Part model, mm, in its own coordinate system. A direction names the side the tool comes from. Coordinates: 2 decimals unless noted, no trailing zeros. Order: outer loops, then holes, each group sorted by start corner. A loop starts at its lowest first (then second) coordinate and runs counter-clockwise, first axis right, second up. Notation, with made-up numbers: (63, 75) - (73, 75) arc R19 ccw to (73, 94) - close; hole circle Ø10 at (11.25, 12.5). An arc over 180 degrees is marked (long way). Use a Markdown table: item, result. Add a question column.
1) Saw through at B-B on z = -28.5. List the corners of the cut face in (x, y), then the cut area to 3 significant figures.
2) Drop flat-ended pins along their axis: P1, Ø14.5, axis at x = 54.5, y = -42.5, coming from the -Z side; P2, Ø12, axis at y = -70.5, z = -56.5, coming from the -X side; P3, Ø12, axis at y = -11.5, z = -26, coming from the -X side. Give the stop position or say it passes through.
3) Saw through at D-D on x = 12. List the corners of the cut face in (y, z), then the cut area to 3 significant figures.
4) Tool access for faces 1 (the face through (37.1, -19.76, -46.64)), 2 (the face through (49, 0, -37)), 3 (the face through (90, -142, 10)), 4 (the face through (0, -74, 10)), 5 (the face through (90, -20, -45)): list every direction of +Z, -Z, +X, -X, +Y, -Y with a clear straight run to the whole face (end or side of a thin tool).
5) Two-plate mould, pull along Y, no slides. Class faces 6 (the face through (10, -20, -45)), 7 (the face through (49.93, -95.495, -46.644)), 8 (the face through (50, -40, 0)): +Y half, -Y half, draft (parallel to the pull), parting line (faces both ways), or undercut.
6) Saw through at A-A on y = -138.5. List the corners of the cut face in (x, z).
7) Saw through at C-C on y = -30. List the corners of the cut face in (x, z), then the cut area to 3 significant figures.
8) Wall check: L1, parallel to X at y = -6, z = -82; L2, parallel to Z at x = 83, y = -73; L3, parallel to Y at x = 49, z = -75.5. Give the ranges that are in metal, low to high. Write a range as [from, to].
```python
from build123d import *

# Parameters (mm, degrees)
BASE_PLATE_20MM_DEPTH   = 20
BLOCK_92MM_DEPTH        = 92
RELIEF_CUT_SKETCH_R     = 24
RELIEF_CUT_DEPTH        = 92
GUSSET_100MM_DEPTH      = 100
GUSSET_TRIM_CUT_1_DEPTH = 45
GUSSET_TRIM_CUT_2_DEPTH = 45


with BuildPart() as part:
    # Base Plate Sketch → Base Plate 20mm (new body)
    with BuildSketch(Plane.XY):
        Polygon((0, 0), (100, 0), (100, -150), (90, -150), (90, -134), (10, -134), (10, -150), (0, -150), align=None)
    extrude(amount=BASE_PLATE_20MM_DEPTH)

    # Block Sketch → Block 92mm (add)
    with BuildSketch(Plane(origin=(0, 0, 0), x_dir=(-1, 0, 0), z_dir=(0, 0, -1))):
        with BuildLine():
            Line((-10, -40), (-10, 0))
            Line((-10, 0), (-90, 0))
            Line((-90, 0), (-90, -40))
            ThreePointArc((-90, -40), (-50, -80), (-10, -40))
        make_face()
    extrude(amount=BLOCK_92MM_DEPTH)

    # Relief Cut Sketch → Relief Cut (cut)
    with BuildSketch(Plane(origin=(0, 0, -92), x_dir=(-1, 0, 0), z_dir=(0, 0, -1))):
        with Locations((-50, -40)):
            Circle(RELIEF_CUT_SKETCH_R)
    extrude(amount=-RELIEF_CUT_DEPTH, mode=Mode.SUBTRACT)

    # Gusset Sketch → Gusset 100mm (add)
    with BuildSketch(Plane.ZY):
        Polygon((-92, -80), (0, -111.42938948), (0, -79.30503211), align=None)
    extrude(amount=-GUSSET_100MM_DEPTH)

    # Gusset Trim Sketch 1 → Gusset Trim Cut 1 (cut)
    with BuildSketch(Plane.ZY):
        Polygon((-92, -80), (0, -79.30503211), (0, -111.42938948), align=None)
    extrude(amount=-GUSSET_TRIM_CUT_1_DEPTH, mode=Mode.SUBTRACT)

    # Gusset Trim Sketch 2 → Gusset Trim Cut 2 (cut)
    with BuildSketch(Plane(origin=(100, 0, 0), x_dir=(0, 0, -1), z_dir=(1, 0, 0))):
        Polygon((0, -79.30503211), (92, -80), (0, -111.42938948), align=None)
    extrude(amount=-GUSSET_TRIM_CUT_2_DEPTH, mode=Mode.SUBTRACT)


solid = part.part
```
Results are:
| question | item | result |
|---|---|---|
| 1 | outline | (10, -40) arc R40 ccw to (43.82, -79.52) - (45, -79.52) - (45, -101.69) - (55, -101.69) - (55, -79.52) - (56.18, -79.52) arc R40 ccw to (90, -40) - (90, 0) - (10, 0) - close; hole circle Ø48 at (50, -40) |
| 1 | area | 4,120 mm2 |
| 2 | P1 | z = 0 |
| 2 | P2 | x = 18.38 |
| 2 | P3 | x = 10 |
| 3 | outline | (-134, 0) - (-52.49, 0) - (-52.49, -92) - (0, -92) - (0, 20) - (-134, 20) - close |
| 3 | area | 7,510 mm2 |
| 4 | face 1 | -Z |
| 4 | face 2 | +Z, -Z, +X, -X, +Y |
| 4 | face 3 | +Z, -Z, -Y |
| 4 | face 4 | +Z, -Z, -X, +Y, -Y |
| 4 | face 5 | -Z, +X, +Y, -Y |
| 5 | face 6 | draft |
| 5 | face 7 | -Y half |
| 5 | face 8 | undercut |
| 6 | outline | (0, 0) - (10, 0) - (10, 20) - (0, 20) - close; (90, 0) - (100, 0) - (100, 20) - (90, 20) - close |
| 7 | outline | (0, 0) - (10, 0) - (10, -92) - (28.18, -92) - (28.18, 0) - (71.82, 0) - (71.82, -92) - (90, -92) - (90, 0) - (100, 0) - (100, 20) - (0, 20) - close |
| 7 | area | 5,350 mm2 |
| 8 | L1 | [10, 90] |
| 8 | L2 | [0, 20] |
| 8 | L3 | [-85.64, -63.98], [-16.02, 0] |
